from build123d import *

# Parameters (mm, degrees)
SKETCH1_W             = 120
SKETCH1_H             = 40
EXTRUDE1_DEPTH        = 6
M6_TAPPED_HOLE1_D     = 5
M6_TAPPED_HOLE1_DEPTH = 15
M6_TAPPED_HOLE1_TIP   = 1.502151548
CHAMFER1_SIZE         = 5


with BuildPart() as part:
    # Sketch1 → Extrude1 (new, symmetric)
    with BuildSketch(Plane(origin=(0, 0, 0), x_dir=(1, 0, 0), z_dir=(0, 1, 0))):
        Rectangle(SKETCH1_W, SKETCH1_H)
    extrude(amount=EXTRUDE1_DEPTH, both=True)

    # M6 Tapped Hole1
    with Locations(Plane(origin=(0, 6, 0), x_dir=(-1, 0, 0), z_dir=(0, 1, 0))):
        with Locations((40, 0), (-40, 0)):
            Hole(M6_TAPPED_HOLE1_D / 2, depth=M6_TAPPED_HOLE1_DEPTH)
            with Locations((0, 0, -(M6_TAPPED_HOLE1_DEPTH + M6_TAPPED_HOLE1_TIP / 2))):  # 118° drill point
                Cone(0, M6_TAPPED_HOLE1_D / 2, M6_TAPPED_HOLE1_TIP, mode=Mode.SUBTRACT)

    # Chamfer1
    chamfer1_edges = [part.edges().sort_by_distance(p)[0] for p in [
        (-60, 0, -20),
        (60, 0, -20),
        (60, 0, 20),
        (-60, 0, 20),
    ]]
    chamfer(chamfer1_edges, length=CHAMFER1_SIZE)


solid = part.part
The model under review builds one solid part; all positions refer to its coordinate system, in mm. Round coordinates to 2 decimals unless told otherwise and drop trailing zeros. Order: outer loops, then holes, each group sorted by start corner. A loop starts at its lowest first (then second) coordinate and runs counter-clockwise, first axis right, second up. Notation, with made-up numbers: (84, 41.5) -> (90, 41.5) arc R32 ccw to (90, 77.5) -> close; hole circle Ø3 at (-7, 64.25). An arc over 180 degrees is marked (long way). Use CSV: the item, a comma, the result in double quotes. Start each with the question number.
(1) Mouldability with a two-part tool opening along Z and no side actions: class faces 1 (the face through (-1, 0, 20)), 2 (the face through (-37.69, -0.08, -0.96)), 3 (the face through (-1, 0, -20)), 4 (the face through (60, 0, 0)) as pulls with the +Z half, pulls with the -Z half, needs draft (parallel to the pull), parting line crosses it, or undercut.
(2) Consider section C-C on y = -4.5. Write out the cut boundary in (x, z).
(3) Consider section B-B on z = 0. Write out the cut boundary in (x, y), and give its area (3 significant figures).
(4) Wall thickness on probe 1 along Z at (x, y) = (40, -1.5); probe 2 along X at (y, z) = (2.5, 17): over which ranges is each line inside the solid? List them lowest first. Write a range as from..to.
(5) Consider section A-A on x = -40. Write out the cut boundary in (y, z), and give its area (3 significant figures).
Responses:
1,face 1,"pulls with the +Z half"
1,face 2,"undercut"
1,face 3,"pulls with the -Z half"
1,face 4,"needs draft"
2,outline,"(-60, -15) -> (-55, -20) -> (55, -20) -> (60, -15) -> (60, 15) -> (55, 20) -> (-55, 20) -> (-60, 15) -> close; hole circle Ø5 at (-40, 0); hole circle Ø5 at (40, 0)"
3,outline,"(-60, -6) -> (-42.5, -6) -> (-42.5, 6) -> (-60, 6) -> close; (-37.5, -6) -> (37.5, -6) -> (37.5, 6) -> (-37.5, 6) -> close; (42.5, -6) -> (60, -6) -> (60, 6) -> (42.5, 6) -> close"
3,area,"1,320 mm²"
4,probe 1,"-20..-2.5, 2.5..20"
4,probe 2,"-58..58"
5,outline,"(-6, -20) -> (6, -20) -> (6, -2.5) -> (-6, -2.5) -> close; (-6, 2.5) -> (6, 2.5) -> (6, 20) -> (-6, 20) -> close"
5,area,"420 mm²"
